from build123d import *

# Parameters (mm, degrees)
CIRPATTERN1_COUNT = 6
CIRPATTERN2_COUNT = 6


with BuildPart() as part:
    # Sketch1 → Revolve1 (revolve)
    with BuildSketch(Plane.XY, mode=Mode.PRIVATE) as revolve1_sk:
        Polygon((-135, 0), (-135, 53), (-117, 53), (-117, 62), (-76, 62), (-76, 88), (-117, 88), (-117, 97), (-135, 97), (-135, 186), (-300, 186), (-315.79829971, 66), (-185, 66), (-185, 0), align=None)
    revolve(revolve1_sk.sketch.rotate(Axis((0, 0, 0), (0, 1, 0)), 270), axis=Axis((0, 0, 0), (0, 1, 0)))

    # Sketch3 → 1/2-13 Tapped Hole1 (revolve, cut)
    with BuildSketch(Plane(origin=(160, 186, 0), x_dir=(0, 0, 1), z_dir=(1, 0, 0))):
        Polygon((0, 0), (0, 28.619489309), (5.35813, 25.4), (5.35813, 0), align=None)
    f_1_2_13_tapped_hole1 = revolve(axis=Axis((160, 192.35, 0), (0, -1, 0)), mode=Mode.SUBTRACT)

    # CirPattern1: 1/2-13 Tapped Hole1 ×6 about axis
    cirpattern1_axis = Axis((0, 0, 0), (0, 1, 0))
    for i in range(1, CIRPATTERN1_COUNT):
        add(f_1_2_13_tapped_hole1.rotate(cirpattern1_axis, i * 360 / CIRPATTERN1_COUNT), mode=Mode.SUBTRACT)

    # Sketch5 → 1/2-13 Tapped Hole2 (revolve, cut)
    with BuildSketch(Plane(origin=(160, 0, 0), x_dir=(0, 0, -1), z_dir=(1, 0, 0))):
        Polygon((0, 0), (0, 34.479489309), (5.35813, 31.26), (5.35813, 0), align=None)
    f_1_2_13_tapped_hole2 = revolve(axis=Axis((160, -6.35, 0), (0, 1, 0)), mode=Mode.SUBTRACT)

    # CirPattern2: 1/2-13 Tapped Hole2 ×6 about axis
    cirpattern2_axis = Axis((0, 0, 0), (0, 1, 0))
    for i in range(1, CIRPATTERN2_COUNT):
        add(f_1_2_13_tapped_hole2.rotate(cirpattern2_axis, i * 360 / CIRPATTERN2_COUNT), mode=Mode.SUBTRACT)


solid = part.part
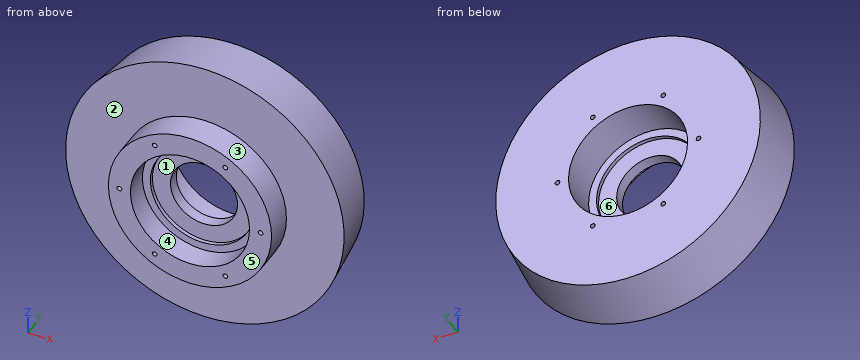
Geometry: final body of the model. Coordinates: model frame, mm. Face numbers are marked on the shaded views. A direction names the side the tool comes from. Give positions to 0.01 mm unless a question says otherwise; leave off trailing zeros. Loops run counter-clockwise (first coordinate to the right, second up) from the corner with the lowest first, then second, coordinate; pieces in that order, holes last. Notation, with made-up numbers: (71.25, -39.5) - (98.25, -39.5) arc R27 ccw to (98.25, -18.5) - close; hole circle Ø11 at (60, 9). An arc over 180 degrees is marked (long way). One line per question, with ' | ' between items. Start each with the question number.
(1) Section query A-A on x = 0. Return loops of the section in (y, z).
(2) Ray query, line 1 (X direction, y = 19, z = 0.5); line 2 (X direction, y = 7, z = 0); line 3 (Y direction, x = 94, z = 226.5). Return the intervals inside material, ascending. Write a range as from..to.
(3) Reachability of the marked faces 4, 5 and 6 from +Z, -Z, +X, -X, +Y, -Y: full face, straight path, thin tool, end or side. Return the list, or none.
(4) Pull-direction query (Z, two-part tool) for the marked faces 1, 2 and 3; classes: released by +Z, released by -Z, zero draft, split by the parting line, or undercut.
(5) Contact query for flat-ended pins moving along their axis: pin 1 (10 mm diameter, centred on y = 43, z = 52, fed in from +X); pin 2 (1.5 mm diameter, centred on x = 151.5, y = 127.5, fed in from -Z); pin 3 (1.5 mm diameter, centred on x = -110, y = 150.5, fed in from -Z); pin 4 (12.5 mm diameter, centred on x = -80, z = 138.56, fed in from +Y). Output: stop coordinate, or through.
(6) Section query B-B on y = 147.5. Return loops of the section in (x, z), then the cut area to 3 significant figures.
The answers:
1) outline: (0, -185) - (66, -185) - (66, -315.8) - (186, -300) - (186, -135) - (97, -135) - (97, -117) - (88, -117) - (88, -76) - (62, -76) - (62, -117) - (53, -117) - (53, -135) - (0, -135) - close; (0, 135) - (53, 135) - (53, 117) - (62, 117) - (62, 76) - (88, 76) - (88, 117) - (97, 117) - (97, 135) - (186, 135) - (186, 300) - (66, 315.8) - (66, 185) - (0, 185) - close
2) line 1: -185..-165.33, -154.67..-135, 135..154.67, 165.33..185 | line 2: -185..-165.36, -154.64..-135, 135..154.64, 165.36..185 | line 3: 66..186
3) face 4: -Y | face 5: +Z, -Z, +X, -X, -Y | face 6: +Y
4) face 1: undercut | face 2: zero draft | face 3: split by the parting line
5) pin 1: x = 178.93 | pin 2: z = -268.26 | pin 3: z = -284.43 | pin 4: y = 186
6) outline: circle Ø610.14 at (0, 0); hole circle Ø270 at (0, 0) | area: 235,000 mm2
